Design review of the part built by this model. Coordinates are the model's own, in mm. A direction names the side the tool comes from. Coordinates: 2 decimals unless noted, no trailing zeros. Loops run counter-clockwise (first coordinate to the right, second up) from the corner with the lowest first, then second, coordinate; pieces in that order, holes last. Notation, with made-up numbers: (55, 73.25) -> (59, 73.25) arc R7 cw to (59, 85.25) -> close; hole circle Ø10 at (87, 68). An arc over 180 degrees is marked (long way). Use CSV: the item, a comma, the result in double quotes.
```python
from build123d import *

# Parameters (mm, degrees)
EXTRUDE_THIN1_DEPTH = 2
FILLET1_R           = 2
FILLET2_R           = 0.5


with BuildPart() as part:
    # Sketch1 → Extrude-Thin1 (new body)
    with BuildSketch(Plane.XY):
        Polygon((0, 0), (0, 8.954475992), (14.596760519, 8.954475992), (14.596760519, 0), (16.596760519, 0), (16.596760519, 10.954475992), (-2, 10.954475992), (-2, 0), align=None)
    extrude(amount=EXTRUDE_THIN1_DEPTH)

    # Fillet1
    fillet1_edges = [part.edges().sort_by_distance(p)[0] for p in [
        (-2, 10.954475992, 1),
        (16.596760519, 10.954475992, 1),
        (14.596760519, 8.954475992, 1),
        (0, 8.954475992, 1),
    ]]
    fillet(fillet1_edges, radius=FILLET1_R)

    # Fillet2
    fillet2_edges = [part.edges().sort_by_distance(p)[0] for p in [
        (16.596760519, 4.477237996, 2),
        (7.29838026, 10.954475992, 0),
        (7.29838026, 10.954475992, 2),
        (-2, 4.477237996, 0),
        (-1.414213562, 10.368689555, 0),
        (16.010974082, 10.368689555, 0),
        (-2, 4.477237996, 2),
        (-1.414213562, 10.368689555, 2),
        (16.010974082, 10.368689555, 2),
        (16.596760519, 4.477237996, 0),
    ]]
    fillet(fillet2_edges, radius=FILLET2_R)


solid = part.part
```
Item 1: Add section A-A (y = 5.25). Give the boundary of the cut face in (x, z).
Checked values:
outline,"(-2, 0.5) arc R0.5 ccw to (-1.5, 0) -> (0, 0) -> (0, 2) -> (-1.5, 2) arc R0.5 ccw to (-2, 1.5) -> close; (14.6, 0) -> (16.1, 0) arc R0.5 ccw to (16.6, 0.5) -> (16.6, 1.5) arc R0.5 ccw to (16.1, 2) -> (14.6, 2) -> close"
Item 2: Machinability: for faces 1 (the face through (16, 0, 1)), 2 (the face through (7, 8.954, 1)), which of the approach directions +Z, -Z, +X, -X, +Y, -Y give a long, thin tool a straight path to every point of the face, cutting with its end or side? Answer none if there is none.
Checked values:
face 1,"+Z, -Z, +X, -X, -Y"
face 2,"+Z, -Z, -Y"
Item 3: Add section C-C (x = 3.25). Give the boundary of the cut face in (y, z), then the cut area to 3 significant figures.
Checked values:
outline,"(8.95, 0) -> (10.45, 0) arc R0.5 ccw to (10.95, 0.5) -> (10.95, 1.5) arc R0.5 ccw to (10.45, 2) -> (8.95, 2) -> close"
area,"3.89 mm^2"
Item 4: Add section D-D (y = 8.5). Give the boundary of the cut face in (x, z).
Checked values:
outline,"(-2, 0.5) arc R0.5 ccw to (-1.5, 0) -> (0.73, 0) -> (0.73, 2) -> (-1.5, 2) arc R0.5 ccw to (-2, 1.5) -> close; (13.87, 0) -> (16.1, 0) arc R0.5 ccw to (16.6, 0.5) -> (16.6, 1.5) arc R0.5 ccw to (16.1, 2) -> (13.87, 2) -> close"
Item 5: To check wall thickness, follow line 1 along X through (y, z) = (4.25, 0.75); line 2 along Y through (x, z) = (2.25, 0.65); line 3 along X through (y, z) = (7.5, 0.5). State the ranges of each line that lie inside material, in increasing order.
Checked values:
line 1,"-2 to 0, 14.6 to 16.6"
line 2,"8.95 to 10.95"
line 3,"-2 to 0.08, 14.52 to 16.6"
Item 6: Add section B-B (z = 1.2). Give the boundary of the cut face in (x, y).
Checked values:
outline,"(-2, 0) -> (0, 0) -> (0, 6.95) arc R2 cw to (2, 8.95) -> (12.6, 8.95) arc R2 cw to (14.6, 6.95) -> (14.6, 0) -> (16.6, 0) -> (16.6, 8.95) arc R2 ccw to (14.6, 10.95) -> (0, 10.95) arc R2 ccw to (-2, 8.95) -> close"
